```python
from build123d import *

# Parameters (mm, degrees)
BOSS_EXTRUDE1_DEPTH = 20
CUT_EXTRUDE1_DEPTH  = 50


with BuildPart() as part:
    # Sketch1 → Boss-Extrude1 (new body)
    with BuildSketch(Plane.XY):
        Polygon((5, 0), (137.6, 0), (142.6, 5), (142.6, 48), (0, 10), (0, 5), align=None)
    extrude(amount=BOSS_EXTRUDE1_DEPTH)

    # Sketch2 → Cut-Extrude1 (cut, along a direction that is not the sketch's normal)
    with BuildSketch(Plane(origin=(-2.488112271, 9.33696868, 0), x_dir=(0.9662799118048497, 0.25749394564224604, 0), z_dir=(-0.257493945642246, 0.9662799118048496, 0))):
        Polygon((150.151224814, 0), (135.474939456, -20), (150.151224814, -20), align=None)
        Polygon((2.574939456, -20), (2.574939456, 0), (9.874939456, -20), align=None)
    extrude(amount=-CUT_EXTRUDE1_DEPTH, dir=(0, 1, 0), mode=Mode.SUBTRACT)


solid = part.part
```
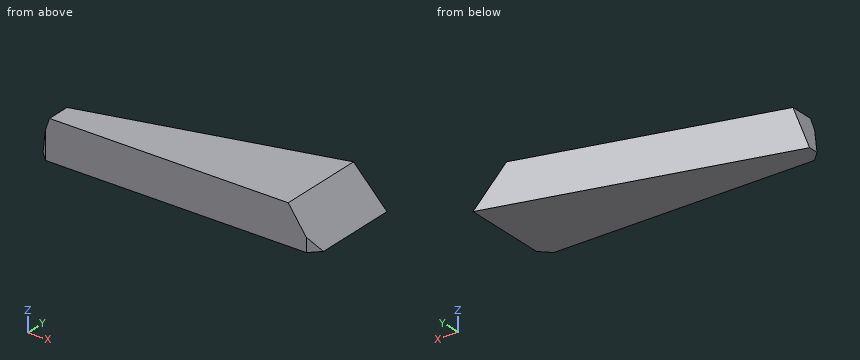
Part model, mm, in its own coordinate system. Round coordinates to 2 decimals unless told otherwise and drop trailing zeros. Write each loop counter-clockwise with the first axis right and the second up, starting at its lowest first coordinate (ties: lowest second). Pieces come first, ordered by that corner, then holes. Notation, with made-up numbers: (-5, 36) -> (41, 36) arc R23 cw to (41, 52) -> close; hole circle Ø3 at (78, -37.5). An arc over 180 degrees is marked (long way). Return JSON: item names as keys, results as strings. Group by question number.
Q1. Saw through at D-D on z = 3.5. Write the cut outline in (x, y), plus the area to 3 significant figures.
Q2. Probe L1, parallel to Y at x = 128.5, z = 2.25; L2, parallel to Y at x = 34, z = 10.75; L3, parallel to Z at x = 133, y = 17.5. List the from-to ranges inside material, lowest first. Write a range as [from, to].
Q3. Saw through at B-B on x = 50.5. Write the cut outline in (y, z), plus the area to 3 significant figures.
Q4. Saw through at C-C on y = 22.5. Write the cut outline in (x, z).
Q5. Saw through at A-A on z = 10.75. Write the cut outline in (x, y), plus the area to 3 significant figures.
Q6. Pin check, flat tip, straight feed: pin 1 (2 mm diameter, centred on y = 17, z = 6, fed in from +X). Stop position of the tip, or through.
Answer:
{
 "1": {"outline": "(1.23, 3.77) -> (5, 0) -> (137.6, 0) -> (140.12, 2.52) -> (140.12, 47.34) -> (1.23, 10.33) -> close", "area": "3,990 mm2"},
 "2": {"L1": "[0, 44.24]", "L2": "[0, 19.06]", "L3": "[0, 13.54]"},
 "3": {"outline": "(0, 0) -> (23.46, 0) -> (23.46, 20) -> (0, 20) -> close", "area": "469 mm2"},
 "4": {"outline": "(46.91, 0) -> (142.6, 0) -> (128.42, 20) -> (46.91, 20) -> close"},
 "5": {"outline": "(3.79, 1.21) -> (5, 0) -> (134.98, 0) -> (134.98, 45.97) -> (3.79, 11.01) -> close", "area": "3,740 mm2"},
 "6": {"pin 1": "x = 139.05"}
}
